CAD build for the part. Positions are in the model's coordinates, mm. A direction names the side the tool comes from. Coordinates: 2 decimals unless noted, no trailing zeros. Order: outer loops, then holes, each group sorted by start corner. A loop starts at its lowest first (then second) coordinate and runs counter-clockwise, first axis right, second up. Notation, with made-up numbers: M 31,67.25 L 35,67.25 A21 ccw 35,82.25 Z; hole C 19,5 d10. An arc over 180 degrees is marked long. Write item = value, one per line. Start each with the question number.
```python
from build123d import *

# Parameters (mm, degrees)
SKETCH1_W           = 40
SKETCH1_H           = 40
BOSS_EXTRUDE1_DEPTH = 30
SKETCH2_W           = 5
SKETCH2_H           = 5
CUT_EXTRUDE1_DEPTH  = 55
SKETCH3_R           = 1.5
CUT_EXTRUDE2_DEPTH  = 55
FILLET1_R           = 2
SKETCH4_R           = 12.5
BOSS_EXTRUDE2_DEPTH = 1
FILLET2_R           = 1
SKETCH5_R           = 5
BOSS_EXTRUDE3_DEPTH = 15


with BuildPart() as part:
    # Sketch1 → Boss-Extrude1 (new, symmetric)
    with BuildSketch(Plane.XY):
        Rectangle(SKETCH1_W, SKETCH1_H)
    extrude(amount=BOSS_EXTRUDE1_DEPTH, both=True)

    # Sketch2 → Cut-Extrude1 (cut)
    with BuildSketch(Plane.XY.offset(30)):
        with Locations((-17.5, 17.5)):
            Rectangle(SKETCH2_W, SKETCH2_H)
        with Locations((17.5, 17.5)):
            Rectangle(SKETCH2_W, SKETCH2_H)
        with Locations((17.5, -17.5)):
            Rectangle(SKETCH2_W, SKETCH2_H)
        with Locations((-17.5, -17.5)):
            Rectangle(SKETCH2_W, SKETCH2_H)
    extrude(amount=-CUT_EXTRUDE1_DEPTH, mode=Mode.SUBTRACT)

    # Sketch3 → Cut-Extrude2 (cut)
    with BuildSketch(Plane.XY.offset(-25)):
        with Locations((-17.5, 17.5)):
            Circle(SKETCH3_R)
        with Locations((17.5, 17.5)):
            Circle(SKETCH3_R)
        with Locations((17.5, -17.5)):
            Circle(SKETCH3_R)
        with Locations((-17.5, -17.5)):
            Circle(SKETCH3_R)
    extrude(amount=-CUT_EXTRUDE2_DEPTH, mode=Mode.SUBTRACT)

    # Fillet1
    fillet1_edges = [part.edges().sort_by_distance(p)[0] for p in [
        (20, -20, -27.5),
        (-20, -20, -27.5),
        (-20, 20, -27.5),
        (20, 20, -27.5),
    ]]
    fillet(fillet1_edges, radius=FILLET1_R)

    # Sketch4 → Boss-Extrude2 (add, symmetric)
    with BuildSketch(Plane.XY.offset(30)):
        Circle(SKETCH4_R)
    extrude(amount=BOSS_EXTRUDE2_DEPTH, both=True)

    # Fillet2
    fillet2_edges = [part.edges().sort_by_distance(p)[0] for p in [
        (-15, -15, 2.5),
        (15, -15, 2.5),
        (15, 15, 2.5),
        (-15, 15, 2.5),
    ]]
    fillet(fillet2_edges, radius=FILLET2_R)

    # Sketch5 → Boss-Extrude3 (add)
    with BuildSketch(Plane(origin=(0, 0, -30), x_dir=(-1, 0, 0), z_dir=(0, 0, -1))):
        with Locations(Location((0, 0, 0), (0, 0, 180))):
            Circle(SKETCH5_R)
    extrude(amount=BOSS_EXTRUDE3_DEPTH)


solid = part.part
```
1. 3-axis set-ups, long thin cutter, end or side, ignore diameter. For faces 4 (the flat face through (-9, 9, 30)), 5 (the flat face through (16, 16, -25)), 6 (the flat face through (16, -16, -25)), 7 (the flat face through (-15, 18, 3)), 8 (the flat face through (-18, -15, 3)): which of +Z, -Z, +X, -X, +Y, -Y reach the whole face in a straight line?
2. Slice it at B-B (z = 19.5). Write the cut outline in (x, y), plus the area to 3 significant figures.
3. Flat gauge pins, fed straight in: pin 1 (2.5 mm diameter, centred on x = -17.5, y = 17.5, fed in from -Z); pin 2 (4.5 mm diameter, centred on y = 19, z = -7.5, fed in from -X); pin 3 (1.2 mm diameter, centred on x = -18.5, z = -1, fed in from +Y); pin 4 (3 mm diameter, centred on y = 17, z = -7.5, fed in from +X). Where does each tip first touch, or does it go through?
4. Slice it at D-D (x = 9). Write the cut outline in (y, z).
5. Probe L1, parallel to Y at x = 17.5, z = -26.05; L2, parallel to X at y = -17, z = -27; L3, parallel to Y at x = 18, z = 22. List the from-to ranges inside material, lowest first.
6. Mould opens along Y. For faces 1 (the flat face through (-15, -18, 3)), 2 (the cylindrical face through (16, 17.57, -27.46)), 3 (the flat face through (0, -20, 0)) say: released by +Y, released by -Y, zero draft, split by the parting line, or undercut.
7. Slice it at A-A (x = 0). Write the cut outline in (y, z).
Calculated:
q1.face_4 = +Z
q1.face_5 = +Z, +X, +Y
q1.face_6 = +Z, +X, -Y
q1.face_7 = +Z, -X, +Y
q1.face_8 = +Z, -X, -Y
q2.outline = M -20,-15 L -16,-15 A1 cw -15,-16 L -15,-20 L 15,-20 L 15,-16 A1 cw 16,-15 L 20,-15 L 20,15 L 16,15 A1 cw 15,16 L 15,20 L -15,20 L -15,16 A1 cw -16,15 L -20,15 Z
q2.area = 1,500 mm²
q3.pin_1 = through
q3.pin_2 = -15
q3.pin_3 = 15
q3.pin_4 = 15.13
q4.outline = M -20,-30 L 20,-30 L 20,30 L 8.67,30 L 8.67,31 L -8.67,31 L -8.67,30 L -20,30 Z
q5.L1 = -20 to -19, -16 to 16, 19 to 20
q5.L2 = -20 to -18.91, -16.09 to 16.09, 18.91 to 20
q5.L3 = -15 to 15
q6.face_1 = zero draft
q6.face_2 = undercut
q6.face_3 = released by -Y
q7.outline = M -20,-30 L -5,-30 L -5,-45 L 5,-45 L 5,-30 L 20,-30 L 20,30 L 12.5,30 L 12.5,31 L -12.5,31 L -12.5,30 L -20,30 Z
